```python
from build123d import *

# Parameters (mm, degrees)
SKETCH_1_W                    = 80
SKETCH_1_H                    = 80
EXTRUDE_1_DEPTH               = 12
CHAMFER_1_SIZE                = 5
HOLE_WIZARD_M12_1_D           = 10.2
HOLE_WIZARD_M12_1_DEPTH       = 32.75
HOLE_WIZARD_M12_1_CSINK_D     = 12.05
HOLE_WIZARD_M12_1_CSINK_ANGLE = 90
HOLE_WIZARD_M12_1_TIP         = 3.064389157


with BuildPart() as part:
    # 草图1 → 凸台-拉伸1 (new body)
    with BuildSketch(Plane.XY):
        Rectangle(SKETCH_1_W, SKETCH_1_H)
    extrude(amount=EXTRUDE_1_DEPTH)

    # 倒角1
    chamfer_1_edges = [part.edges().sort_by_distance(p)[0] for p in [
        (40, -40, 6),
        (-40, -40, 6),
        (-40, 40, 6),
        (40, 40, 6),
    ]]
    chamfer(chamfer_1_edges, length=CHAMFER_1_SIZE)

    # M12 螺纹孔1
    with Locations(Plane(origin=(0, 20, 12), x_dir=(1, 0, 0), z_dir=(0, 0, 1))):
        with Locations((0, 0), (0, -40)):
            CounterSinkHole(HOLE_WIZARD_M12_1_D / 2, HOLE_WIZARD_M12_1_CSINK_D / 2, depth=HOLE_WIZARD_M12_1_DEPTH, counter_sink_angle=HOLE_WIZARD_M12_1_CSINK_ANGLE)
            with Locations((0, 0, -(HOLE_WIZARD_M12_1_DEPTH + HOLE_WIZARD_M12_1_TIP / 2))):  # 118° drill point
                Cone(0, HOLE_WIZARD_M12_1_D / 2, HOLE_WIZARD_M12_1_TIP, mode=Mode.SUBTRACT)


solid = part.part
```
Here's how the part is built. I have some questions about the finished solid (model axes, mm). Round coordinates to 2 decimals unless told otherwise and drop trailing zeros. Order: outer loops, then holes, each group sorted by start corner. A loop starts at its lowest first (then second) coordinate and runs counter-clockwise, first axis right, second up. Notation, with made-up numbers: M 54.5,16 L 83.5,16 A25 ccw 83.5,37 Z; hole C 85.25,59.25 d9. An arc over 180 degrees is marked long. One line per question, with ' | ' between items.
1) I need wall thicknesses on line 1 along Y through (x, z) = (0, 5.75); line 2 along X through (y, z) = (-20, 8.25); line 3 along X through (y, z) = (22, 7.5). Which ranges of each line are inside material? Lowest first, please.
Working result:
line 1: -40 to -25.1, -14.9 to 14.9, 25.1 to 40 | line 2: -40 to -5.1, 5.1 to 40 | line 3: -40 to -4.69, 4.69 to 40
2) I want a section at C-C, the plane z = 3.75. Write out the boundary of the cut face in (x, y).
Working result:
outline: M -40,-35 L -35,-40 L 35,-40 L 40,-35 L 40,35 L 35,40 L -35,40 L -40,35 Z; hole C 0,-20 d10.2; hole C 0,20 d10.2
3) I want a section at B-B, the plane x = 0. Write out the boundary of the cut face in (y, z) (3 decimals), then the cut area to 3 significant figures.
Working result:
outline: M -40,0 L -25.1,0 L -25.1,11.075 L -26.025,12 L -40,12 Z; M -14.9,0 L 14.9,0 L 14.9,11.075 L 13.975,12 L -13.975,12 L -14.9,11.075 Z; M 25.1,0 L 40,0 L 40,12 L 26.025,12 L 25.1,11.075 Z | area: 713 mm²
4) I want a section at A-A, the plane y = -20. Write out the boundary of the cut face in (x, z) (3 decimals), then the cut area to 3 significant figures.
Working result:
outline: M -40,0 L -5.1,0 L -5.1,11.075 L -6.025,12 L -40,12 Z; M 5.1,0 L 40,0 L 40,12 L 6.025,12 L 5.1,11.075 Z | area: 837 mm²
5) If we mould it in two halves opening along X, with no side actions, what happens to faces 1 (the face through (-1, 1, 12)), 2 (the face through (38, -37, 6)), 3 (the face through (1, 15, 5))? For each: +X half, -X half, draft (parallel to the pull), parting line (faces both ways), or undercut.
Working result:
face 1: draft | face 2: +X half | face 3: undercut
